Part model, mm, in its own coordinate system. A direction names the side the tool comes from. Coordinates: 2 decimals unless noted, no trailing zeros. Order: outer loops, then holes, each group sorted by start corner. A loop starts at its lowest first (then second) coordinate and runs counter-clockwise, first axis right, second up.
from build123d import *

# Parameters (mm, degrees)
BOSS_EXTRUDE1_DEPTH = 10
SKETCH2_R           = 15
BOSS_EXTRUDE2_DEPTH = 80


with BuildPart() as part:
    # Sketch1 → Boss-Extrude1 (new body)
    with BuildSketch(Plane.XY):
        Polygon((17.346513547, 10.364931312), (-0.303037051, 20.204987055), (-17.649550598, 9.840055742), (-17.346513547, -10.364931312), (0.303037051, -20.204987055), (17.649550598, -9.840055742), align=None)
    extrude(amount=BOSS_EXTRUDE1_DEPTH)

    # Sketch2 → Boss-Extrude2 (add)
    with BuildSketch(Plane.XY.offset(10)):
        Circle(SKETCH2_R)
    extrude(amount=BOSS_EXTRUDE2_DEPTH)


solid = part.part
Q1. Cut at D-D on z = 69. Write the cut outline in (x, y), and give its area (3 significant figures).
Results list:
outline: circle Ø30 at (0, 0)
area: 707 mm2
Q2. Cut at A-A on x = -8.5. Write the cut outline in (y, z).
Results list:
outline: (-15.3, 0) - (15.31, 0) - (15.31, 10) - (12.36, 10) - (12.36, 90) - (-12.36, 90) - (-12.36, 10) - (-15.3, 10) - close
Q3. Which spindle directions (+Z, -Z, +X, -X, +Y, -Y) get a long thin tool onto all of the face, cutting with end or side? Do faces 1 (the face through (0, 0, 90)), 2 (the face through (-14.5, -4.4, 10)). Say none if no direction does.
Results list:
face 1: +Z, +X, -X, +Y, -Y
face 2: +Z
Q4. Cut at C-C on z = 8. Write the cut outline in (x, y).
Results list:
outline: (-17.65, 9.84) - (-17.35, -10.36) - (0.3, -20.2) - (17.65, -9.84) - (17.35, 10.36) - (-0.3, 20.2) - close
Q5. Cut at B-B on y = 8. Write the cut outline in (x, z).
Results list:
outline: (-17.62, 0) - (17.38, 0) - (17.38, 10) - (12.69, 10) - (12.69, 90) - (-12.69, 90) - (-12.69, 10) - (-17.62, 10) - close
Q6. Pin check, flat tips, straight feed: pin 1 Ø10 at (x, z) = (5, 55.5) entering from +Y; pin 2 Ø12 at (x, z) = (8, 32.5) entering from +Y; pin 3 Ø3 at (x, z) = (4, 73) entering from +Y. Stop position of each tip, or through.
Results list:
pin 1: stops at y = 15
pin 2: stops at y = 14.87
pin 3: stops at y = 14.79
Q7. Wall check: line 1 along Y through (x, z) = (0.5, 69); line 2 along Z through (x, y) = (12.5, -12); line 3 along X through (y, z) = (-8.5, 27.5). Give the ranges that are in metal, low to high.
Results list:
line 1: y = -14.99 to 14.99
line 2: z = 0 to 10
line 3: x = -12.36 to 12.36
